from build123d import *

# Parameters (mm, degrees)
SKETCH1_R           = 10
BOSS_EXTRUDE1_DEPTH = 30
SKETCH2_R           = 5
BOSS_EXTRUDE2_DEPTH = 20
CHAMFER1_SIZE       = 2
CHAMFER2_SIZE       = 1


with BuildPart() as part:
    # Sketch1 → Boss-Extrude1 (new body)
    with BuildSketch(Plane(origin=(0, 0, 0), x_dir=(1, 0, 0), z_dir=(0, 1, 0))):
        with Locations(Location((0, 0, 0), (0, 0, 270))):
            Circle(SKETCH1_R)
    extrude(amount=BOSS_EXTRUDE1_DEPTH)

    # Sketch2 → Boss-Extrude2 (add)
    with BuildSketch(Plane(origin=(0, 30, 0), x_dir=(1, 0, 0), z_dir=(0, 1, 0))):
        with Locations(Location((0, 0, 0), (0, 0, 270))):
            Circle(SKETCH2_R)
    extrude(amount=BOSS_EXTRUDE2_DEPTH)

    # Chamfer1
    chamfer1_edges = [part.edges().sort_by_distance(p)[0] for p in [
        (0, 0, -10),
    ]]
    chamfer(chamfer1_edges, length=CHAMFER1_SIZE)

    # Chamfer2
    chamfer2_edges = [part.edges().sort_by_distance(p)[0] for p in [
        (0, 50, -5),
    ]]
    chamfer(chamfer2_edges, length=CHAMFER2_SIZE)


solid = part.part
Read the model definition and answer for the solid it produces. Units are mm, in the model's axes. A direction names the side the tool comes from. Give positions to 0.01 mm unless a question says otherwise; leave off trailing zeros. Write each loop counter-clockwise with the first axis right and the second up, starting at its lowest first coordinate (ties: lowest second). Pieces come first, ordered by that corner, then holes. Notation, with made-up numbers: (-34.75, -32.5) - (14.25, -32.5) arc R8 cw to (14.25, -28.5) - close; hole circle Ø3 at (17.5, 8). An arc over 180 degrees is marked (long way). Use CSV: the item, a comma, the result in double quotes. Start each with the question number.
(1) Find section A-A (x = 0). Give the vertices of the cut face in (y, z), plus the area to 3 significant figures.
(2) Given P1, Ø1.5, axis at x = 1.5, y = 11.5, coming from the +Z side; P2, Ø6, axis at x = 7, y = 27.5, coming from the +Z side; P3, Ø2, axis at x = -3, z = 5.5, coming from the +Y side; P4, Ø1.5, axis at y = 43, z = 7.5, coming from the -X side, each flat-ended and moving along its own axis, determine where each tip first touches the part or whether it passes through.
(3) Find section C-C (y = 43.5). Give the vertices of the cut face in (x, z).
(4) Find section B-B (z = 0). Give the vertices of the cut face in (x, y), plus the area to 3 significant figures.
(5) Consider line 1 along Y through (x, z) = (-1, 6); line 2 along X through (y, z) = (30.5, -0.25); line 3 along X through (y, z) = (3.5, 0.25). Determine where each line is inside the solid, lowest interval first.
(6) Find section D-D (y = 13). Give the vertices of the cut face in (x, z).
(7) For faces 1 (the flat face through (0, 50, 0)), 2 (the cylindrical face through (-4.88, 39.37, -1.08)), determine the directions among +Z, -Z, +X, -X, +Y, -Y from which every point of the face is accessible in a straight line to the end or side of a thin tool.
Findings below:
1,outline,"(0, -8) - (2, -10) - (30, -10) - (30, -5) - (49, -5) - (50, -4) - (50, 4) - (49, 5) - (30, 5) - (30, 10) - (2, 10) - (0, 8) - close"
1,area,"795 mm2"
2,P1,"z = 9.97"
2,P2,"z = 9.17"
2,P3,"y = 30"
2,P4,"through"
3,outline,"circle Ø10 at (0, 0)"
4,outline,"(-10, 2) - (-8, 0) - (8, 0) - (10, 2) - (10, 30) - (5, 30) - (5, 49) - (4, 50) - (-4, 50) - (-5, 49) - (-5, 30) - (-10, 30) - close"
4,area,"795 mm2"
5,line 1,"0 to 30"
5,line 2,"-4.99 to 4.99"
5,line 3,"-10 to 10"
6,outline,"circle Ø20 at (0, 0)"
7,face 1,"+Z, -Z, +X, -X, +Y"
7,face 2,"+Y"
